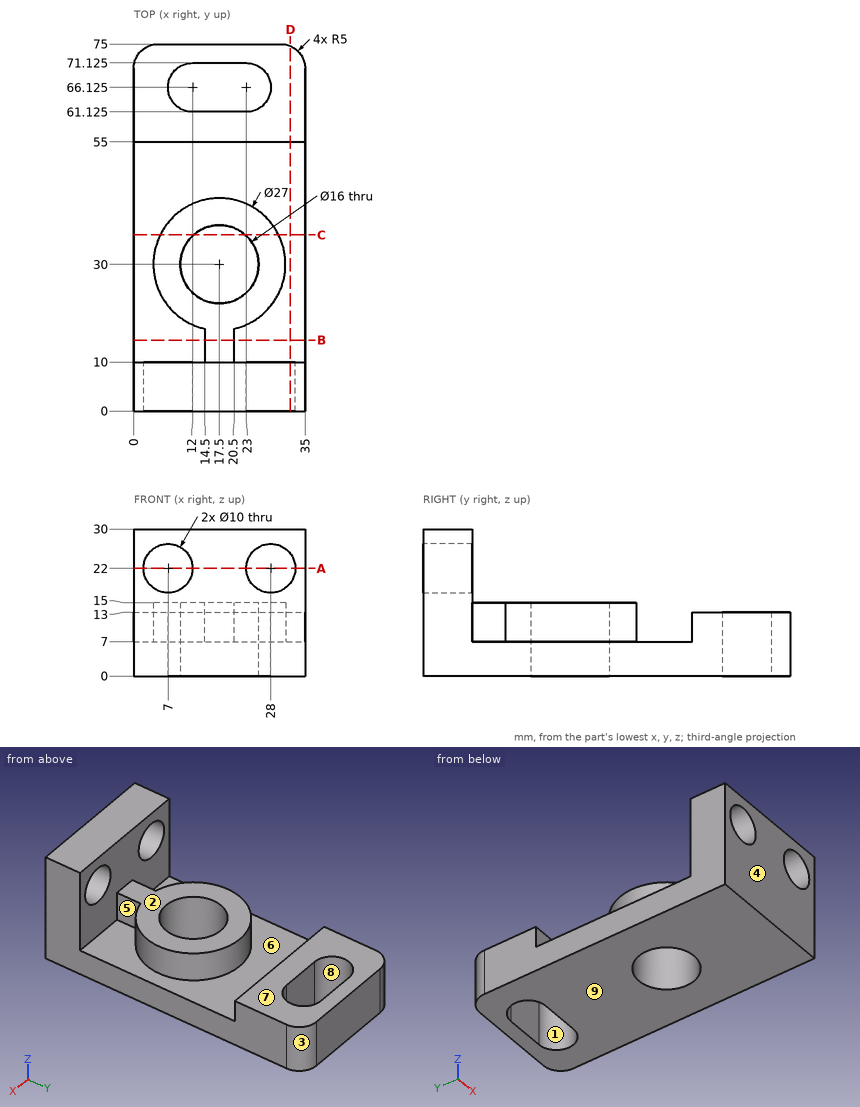
The drawing under review shows one solid part. Ordinate dimensions are in mm from its lowest x, y, z. A direction names the side the tool comes from. Give positions to 0.01 mm unless a question says otherwise; leave off trailing zeros. Order: outer loops, then holes, each group sorted by start corner. A loop starts at its lowest first (then second) coordinate and runs counter-clockwise, first axis right, second up. Notation, with made-up numbers: (42.5, 52) - (91.5, 52) arc R16 cw to (91.5, 61) - close; hole circle Ø2 at (60, 25.5). An arc over 180 degrees is marked (long way). Answer as a JSON object with one key per item and string values. Group by question number.
Item 1: Take a section at C-C on y = 36. Give the boundary of the cut face in (x, z).
Item 2: Machinability: for the marked faces 5, 6, 7, 8 and 9, which of the approach directions +Z, -Z, +X, -X, +Y, -Y give a long, thin tool a straight path to every point of the face, cutting with its end or side? Answer none if there is none.
Item 3: Clearance check with flat-ended pins moving along their axes: pin 1 Ø3.5 at (x, z) = (17, 3.5) entering from -Y; pin 2 Ø10 at (x, y) = (11.5, 67.5) entering from +Z; pin 3 Ø1.5 at (y, z) = (22.5, 14) entering from +X; pin 4 Ø2 at (y, z) = (13.5, 10) entering from -X. State where each tip first meets the part, or that it passes through.
Item 4: Draft analysis for pull direction Y (two halves, no side actions). For the marked faces 1, 2, 3 and 4, state which applies: pulls with the +Y half, pulls with the -Y half, needs draft (parallel to the pull), parting line crosses it, or undercut.
Item 5: Take a section at A-A on z = 22. Give the boundary of the cut face in (x, y), and give its area (3 significant figures).
Item 6: Wall thickness on line 1 along X through (y, z) = (3.25, 22); line 2 along Y through (x, z) = (17.5, 6.25) (3 decimals); line 3 along Y through (x, z) = (17.5, 7.75) (3 decimals): over which ranges is each line inside the solid? List them lowest first.
Item 7: Take a section at D-D on x = 32. Give the boundary of the cut face in (y, z), and give its area (3 significant figures).
Item 8: Take a section at B-B on y = 14.5. Give the boundary of the cut face in (x, z), and give its area (3 significant figures).
Reported:
{
 "1": {"outline": "(0, 0) - (12.21, 0) - (12.21, 15) - (5.41, 15) - (5.41, 7) - (0, 7) - close; (22.79, 0) - (35, 0) - (35, 7) - (29.59, 7) - (29.59, 15) - (22.79, 15) - close"},
 "2": {"face 5": "+Z, +X", "face 6": "+Z", "face 7": "+Z, +X, -X, +Y", "face 8": "+Z, -Z", "face 9": "-Z, +X, -X, +Y, -Y"},
 "3": {"pin 1": "y = 0", "pin 2": "z = 13", "pin 3": "x = 29.19", "pin 4": "x = 14.5"},
 "4": {"face 1": "undercut", "face 2": "needs draft", "face 3": "pulls with the +Y half", "face 4": "pulls with the -Y half"},
 "5": {"outline": "(0, 0) - (2, 0) - (2, 10) - (0, 10) - close; (12, 0) - (23, 0) - (23, 10) - (12, 10) - close; (33, 0) - (35, 0) - (35, 10) - (33, 10) - close", "area": "150 mm^2"},
 "6": {"line 1": "0 to 2, 12 to 23, 33 to 35", "line 2": "0 to 22, 38 to 61.125, 71.125 to 75", "line 3": "0 to 22, 38 to 43.5, 55 to 61.125, 71.125 to 75"},
 "7": {"outline": "(0, 0) - (74.58, 0) - (74.58, 13) - (55, 13) - (55, 7) - (10, 7) - (10, 19) - (0, 19) - close; (0, 25) - (10, 25) - (10, 30) - (0, 30) - close", "area": "810 mm^2"},
 "8": {"outline": "(0, 0) - (35, 0) - (35, 7) - (20.5, 7) - (20.5, 15) - (14.5, 15) - (14.5, 7) - (0, 7) - close", "area": "293 mm^2"}
}
